Work out the finished part from the listing and answer in its coordinate system (mm). A direction names the side the tool comes from. Coordinates: 2 decimals unless noted, no trailing zeros. Loops run counter-clockwise (first coordinate to the right, second up) from the corner with the lowest first, then second, coordinate; pieces in that order, holes last. Notation, with made-up numbers: M 43,0.25 L 64,0.25 A31 cw 64,34.25 Z; hole C -3.75,3.5 d5. An arc over 180 degrees is marked long. Write each question's results on one line, items separated by ' | '.
```python
from build123d import *

# Parameters (mm, degrees)
SKETCH1_W           = 520
SKETCH1_H           = 200
BOSS_EXTRUDE1_DEPTH = 16


with BuildPart() as part:
    # Sketch1 → Boss-Extrude1 (new body)
    with BuildSketch(Plane.XY):
        with Locations((154.849239326, 69.96508599)):
            Rectangle(SKETCH1_W, SKETCH1_H)
        with BuildLine():
            Line((345.350111085, 9.96508599), (214.849239326, 9.96508599))
            ThreePointArc((214.849239326, 9.96508599), (207.778171514, 12.894018179), (204.849239326, 19.96508599))
            Line((204.849239326, 19.96508599), (204.849239326, 119.96508599))
            ThreePointArc((204.849239326, 119.96508599), (207.778171514, 127.036153802), (214.849239326, 129.96508599))
            Line((214.849239326, 129.96508599), (359.849239326, 129.96508599))
            ThreePointArc((359.849239326, 129.96508599), (366.920307138, 127.036153802), (369.849239326, 119.96508599))
            Line((369.849239326, 119.96508599), (369.849239326, 19.96508599))
            ThreePointArc((369.849239326, 19.96508599), (366.920307138, 12.894018179), (359.849239326, 9.96508599))
            Line((359.849239326, 9.96508599), (345.350111085, 9.96508599))
        make_face(mode=Mode.SUBTRACT)
        with BuildLine():
            Line((104.849239326, 19.96508599), (104.849239326, 119.96508599))
            ThreePointArc((104.849239326, 119.96508599), (101.920307138, 127.036153802), (94.849239326, 129.96508599))
            Line((94.849239326, 129.96508599), (-50.150760674, 129.96508599))
            ThreePointArc((-50.150760674, 129.96508599), (-57.221828486, 127.036153802), (-60.150760674, 119.96508599))
            Line((-60.150760674, 119.96508599), (-60.150760674, 19.96508599))
            ThreePointArc((-60.150760674, 19.96508599), (-57.221828486, 12.894018179), (-50.150760674, 9.96508599))
            Line((-50.150760674, 9.96508599), (-35.651632433, 9.96508599))
            Line((-35.651632433, 9.96508599), (94.849239326, 9.96508599))
            ThreePointArc((94.849239326, 9.96508599), (101.920307138, 12.894018179), (104.849239326, 19.96508599))
        make_face(mode=Mode.SUBTRACT)
    extrude(amount=BOSS_EXTRUDE1_DEPTH)


solid = part.part
```
1) Straight lines are drawn through the part: probe 1 along X at (y, z) = (93, 2.25); probe 2 along Y at (x, z) = (17, 7.25); probe 3 along Y at (x, z) = (209.5, 3.5). For each, find the intervals that lie inside material, in ascending order. Write a range as [from, to].
Check result:
probe 1: [-105.15, -60.15], [104.85, 204.85], [369.85, 414.85] | probe 2: [-30.03, 9.97], [129.97, 169.97] | probe 3: [-30.03, 11.52], [128.41, 169.97]
2) Which of the six approach directions +Z, -Z, +X, -X, +Y, -Y give full straight-line access (tool end or side, diameter ignored) to faces 1 (the face through (204.849, 69, 8)), 2 (the face through (-105.151, 69, 8))?
Check result:
face 1: +Z, -Z | face 2: +Z, -Z, -X, +Y, -Y
3) Find section A-A, the plane y = 47. Give the vertices of the cut face in (x, z), and give its area (3 significant figures).
Check result:
outline: M -105.15,0 L -60.15,0 L -60.15,16 L -105.15,16 Z; M 104.85,0 L 204.85,0 L 204.85,16 L 104.85,16 Z; M 369.85,0 L 414.85,0 L 414.85,16 L 369.85,16 Z | area: 3,040 mm^2
4) For a pull along X with two mould halves and no side action, classify faces 3 (the face through (151, 71, 16)), 4 (the face through (-57.299, 12.972, 7.888)), 5 (the face through (414.849, 69, 8)) as released by +X, released by -X, zero draft, split by the parting line, or undercut.
Check result:
face 3: zero draft | face 4: undercut | face 5: released by +X
5) Find section C-C, the plane z = 2.75. Give the vertices of the cut face in (x, y), and give its area (3 significant figures).
Check result:
outline: M -105.15,-30.03 L 414.85,-30.03 L 414.85,169.97 L -105.15,169.97 Z; hole M -60.15,19.97 A10 ccw -50.15,9.97 L 94.85,9.97 A10 ccw 104.85,19.97 L 104.85,119.97 A10 ccw 94.85,129.97 L -50.15,129.97 A10 ccw -60.15,119.97 Z; hole M 204.85,19.97 A10 ccw 214.85,9.97 L 359.85,9.97 A10 ccw 369.85,19.97 L 369.85,119.97 A10 ccw 359.85,129.97 L 214.85,129.97 A10 ccw 204.85,119.97 Z | area: 64,600 mm^2
6) Find section B-B, the plane x = 345. Give the vertices of the cut face in (y, z).
Check result:
outline: M -30.03,0 L 9.97,0 L 9.97,16 L -30.03,16 Z; M 129.97,0 L 169.97,0 L 169.97,16 L 129.97,16 Z
